from build123d import *

# Parameters (mm, degrees)
EXTRUDE_1_DEPTH     = 8
SKETCH_2_R          = 10
CUT_EXTRUDE_1_DEPTH = 8


with BuildPart() as part:
    # 草图1 → 凸台-拉伸1 (new body)
    with BuildSketch(Plane.XY):
        with BuildLine():
            Line((218.63706763, 29.969024264), (0, 25))
            ThreePointArc((0, 25), (-25, 0), (0, -25))
            Line((0, -25), (218.63706763, -29.969024264))
            ThreePointArc((218.63706763, -29.969024264), (190, 0), (218.63706763, 29.969024264))
        make_face()
    extrude(amount=EXTRUDE_1_DEPTH)

    # 草图2 → 切除-拉伸1 (cut)
    with BuildSketch(Plane.XY.offset(8)):
        Circle(SKETCH_2_R)
    extrude(amount=-CUT_EXTRUDE_1_DEPTH, mode=Mode.SUBTRACT)


solid = part.part
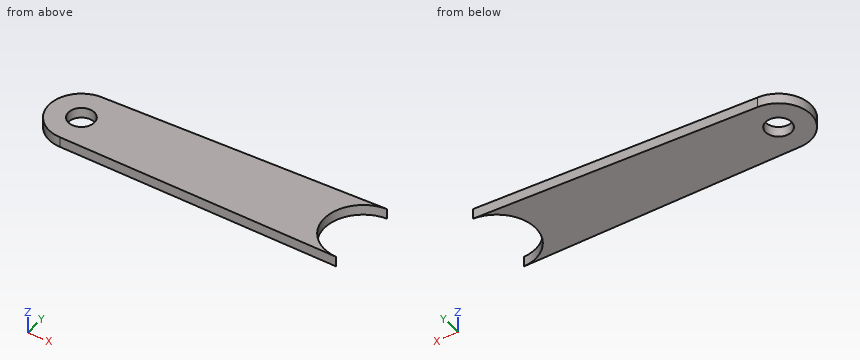
Design review of the part built by this model. Coordinates are the model's own, in mm. Give positions to 0.01 mm unless a question says otherwise; leave off trailing zeros. Loops run counter-clockwise (first coordinate to the right, second up) from the corner with the lowest first, then second, coordinate; pieces in that order, holes last. Notation, with made-up numbers: (46.5, 29) - (90.5, 29) arc R18 cw to (90.5, 47) - close; hole circle Ø4 at (78, -20.75). An arc over 180 degrees is marked (long way). Use CSV: the item, a comma, the result in double quotes. Start each with the question number.
1. Add section D-D (x = 92). State the section outline as (y, z) points, plus the area to 3 significant figures.
2. Wall thickness on L1, parallel to Y at x = 0, z = 3; L2, parallel to X at y = 7, z = 2.75; L3, parallel to X at y = 2.5, z = 5: over which ranges is each line inside the solid? List them lowest first.
3. Add section C-C (x = 30). State the section outline as (y, z) points, plus the area to 3 significant figures.
4. Add section A-A (y = 0). State the section outline as (x, z) points, plus the area to 3 significant figures.
5. Insertion check: P1, Ø2, axis at y = -2, z = 4, coming from the +X side; P2, Ø18, axis at x = 0, y = 0, coming from the +Z side; P3, Ø2, axis at y = 23.5, z = 7, coming from the +X side. Each pin has a flat end and moves straight along its axis. Give the tip position at first contact, or say it passes through.
6. Add section B-B (z = 1.25). State the section outline as (x, y) points.
Results found:
1,outline,"(-27.09, 0) - (27.09, 0) - (27.09, 8) - (-27.09, 8) - close"
1,area,"433 mm²"
2,L1,"y = -25 to -10, 10 to 25"
2,L2,"x = -24 to -7.14, 7.14 to 190.83"
2,L3,"x = -24.87 to -9.68, 9.68 to 190.1"
3,outline,"(-25.68, 0) - (25.68, 0) - (25.68, 8) - (-25.68, 8) - close"
3,area,"411 mm²"
4,outline,"(-25, 0) - (-10, 0) - (-10, 8) - (-25, 8) - close; (10, 0) - (190, 0) - (190, 8) - (10, 8) - close"
4,area,"1,560 mm²"
5,P1,"stops at x = 190.15"
5,P2,"passes through"
5,P3,"stops at x = 202.69"
6,outline,"(0, -25) - (218.64, -29.97) arc R30 cw to (218.64, 29.97) - (0, 25) arc R25 ccw to start; hole circle Ø20 at (0, 0)"
